```python
from build123d import *

# Parameters (mm, degrees)
BOSS_EXTRUDE1_DEPTH = 6
SKETCH2_R           = 4.5
CUT_EXTRUDE1_DEPTH  = 6
CHAMFER1_SIZE       = 20
CHAMFER2_SIZE       = 20


with BuildPart() as part:
    # Sketch1 → Boss-Extrude1 (new body)
    with BuildSketch(Plane(origin=(0, 0, 0), x_dir=(1, 0, 0), z_dir=(0, 1, 0))):
        Polygon((-18.076923077, 61.923076923), (81.923076923, 61.923076923), (81.923076923, -18.076923077), (51.923076923, -18.076923077), (51.923076923, 31.923076923), (-18.076923077, 31.923076923), align=None)
    extrude(amount=BOSS_EXTRUDE1_DEPTH)

    # Sketch2 → Cut-Extrude1 (cut)
    with BuildSketch(Plane(origin=(0, 6, 0), x_dir=(1, 0, 0), z_dir=(0, 1, 0))):
        with Locations(Location((66.923076923, -3.076923077, 0), (0, 0, 270))):
            Circle(SKETCH2_R)
    extrude(amount=-CUT_EXTRUDE1_DEPTH, mode=Mode.SUBTRACT)

    # Chamfer1
    chamfer1_edges = [part.edges().sort_by_distance(p)[0] for p in [
        (-18.076923077, 3, -61.923076923),
    ]]
    chamfer(chamfer1_edges, length=CHAMFER1_SIZE)

    # Chamfer2
    chamfer2_edges = [part.edges().sort_by_distance(p)[0] for p in [
        (81.923076923, 3, -61.923076923),
    ]]
    chamfer(chamfer2_edges, length=CHAMFER2_SIZE)


solid = part.part
```
Check sheet for the modelled part. Datum: model origin and axes. Units: mm. A direction names the side the tool comes from. Coordinates: 2 decimals unless noted, no trailing zeros. Order: outer loops, then holes, each group sorted by start corner. A loop starts at its lowest first (then second) coordinate and runs counter-clockwise, first axis right, second up. Notation, with made-up numbers: (23.5, 61) -> (52.5, 61) arc R35 cw to (52.5, 95) -> close; hole circle Ø3 at (37, -1). An arc over 180 degrees is marked (long way). Write each question's results on one line, items separated by ' | '. Start each with the question number.
1) Material ranges on line 1 along Z through (x, y) = (51, 4); line 2 along X through (y, z) = (2, -6); line 3 along Z through (x, y) = (70, 4.75), recorded low to high.
2) Section check D-D (x = -5.5). Enter the section's corners in (y, z), and give its area (3 significant figures).
3) Depth check by flat-ended pin: pin 1 (1.5 mm diameter, centred on x = 15.5, y = 5, fed in from +Z); pin 2 (3 mm diameter, centred on y = 2.5, z = -8, fed in from -X); pin 3 (1.5 mm diameter, centred on x = 71, y = 2, fed in from -Z). Enter the tip coordinate at first touch or a pass-through.
4) Section check A-A (y = 2). Enter the section's corners in (x, z), and give its area (3 significant figures).
5) Draft check along Z on faces 1 (the face through (-18.077, 3, -37)), 2 (the face through (17, 3, -31.923)), 3 (the face through (71.385, 3.042, 2.491)), 4 (the face through (72.063, 2.958, -51.783)). Enter one of: pulls with the +Z half, pulls with the -Z half, needs draft (parallel to the pull), parting line crosses it, or undercut.
6) Section check B-B (x = 70). Enter the section's corners in (y, z).
7) Section check C-C (z = -4.5). Enter the section's corners in (x, y).
8) Set-up check for faces 5 (the face through (81.923, 3, -12)), 6 (the face through (51.923, 3, -7)): record each of +Z, -Z, +X, -X, +Y, -Y from which the full face is reachable in a straight line by a thin tool's end or side.
Checked values:
1) line 1: -61.92 to -31.92 | line 2: 51.92 to 81.92 | line 3: -53.85 to -0.21, 6.36 to 18.08
2) outline: (0, -54.5) -> (6, -54.5) -> (6, -31.92) -> (0, -31.92) -> close | area: 135 mm²
3) pin 1: z = -31.92 | pin 2: x = 51.92 | pin 3: z = -53.6
4) outline: (-18.08, -41.92) -> (1.92, -61.92) -> (61.92, -61.92) -> (81.92, -41.92) -> (81.92, 18.08) -> (51.92, 18.08) -> (51.92, -31.92) -> (-18.08, -31.92) -> close; hole circle Ø9 at (66.92, 3.08) | area: 4,040 mm²
5) face 1: needs draft | face 2: pulls with the +Z half | face 3: undercut | face 4: pulls with the -Z half
6) outline: (0, -53.85) -> (6, -53.85) -> (6, -0.21) -> (0, -0.21) -> close; (0, 6.36) -> (6, 6.36) -> (6, 18.08) -> (0, 18.08) -> close
7) outline: (51.92, 0) -> (81.92, 0) -> (81.92, 6) -> (51.92, 6) -> close
8) face 5: +Z, -Z, +X, +Y, -Y | face 6: +Z, -X, +Y, -Y
